Can you work these out from the model? Positions are in its coordinate system, mm. A direction names the side the tool comes from. Coordinates: 2 decimals unless noted, no trailing zeros. Write each loop counter-clockwise with the first axis right and the second up, starting at its lowest first coordinate (ties: lowest second). Pieces come first, ordered by that corner, then holes. Notation, with made-up numbers: (21.5, 69) - (27.5, 69) arc R16 cw to (27.5, 87) - close; hole circle Ø9 at (33, -13). An arc over 180 degrees is marked (long way). One line per question, with ' | ' between items. Start each with the question number.
from build123d import *

# Parameters (mm, degrees)
CUT_EXTRUDE_1_DEPTH = 4
SKETCH_3_R          = 15
SKETCH_3_R_2        = 14.3
CUT_EXTRUDE_3_DEPTH = 1.3


with BuildPart() as part:
    # 草图1 → 旋转1 (revolve)
    with BuildSketch(Plane.XY):
        Polygon((0, 0), (0, 17.5), (50, 17.5), (50, 20), (85, 20), (85, 60), (935, 60), (935, 20), (970, 20), (970, 17.5), (1111.3, 17.5), (1111.3, 15), (1154.3, 15), (1154.3, 0), align=None)
    revolve(axis=Axis((1154.3, 0, 0), (-1, 0, 0)))

    # 草图2 → 切除-拉伸1 (cut)
    with BuildSketch(Plane(origin=(0, 15, 0), x_dir=(1, 0, 0), z_dir=(0, 1, 0))):
        with BuildLine():
            Line((1121.3, 4), (1164.3, 4))
            Line((1164.3, 4), (1164.3, -4))
            Line((1164.3, -4), (1121.3, -4))
            ThreePointArc((1121.3, -4), (1117.3, 0), (1121.3, 4))
        make_face()
    extrude(amount=-CUT_EXTRUDE_1_DEPTH, mode=Mode.SUBTRACT)

    # 草图3 → 切除-拉伸3 (cut)
    with BuildSketch(Plane(origin=(1144.5, 0, 0), x_dir=(0, 0, -1), z_dir=(1, 0, 0))):
        with Locations(Location((0, 0, 0), (0, 0, 90))):
            Circle(SKETCH_3_R)
        Circle(SKETCH_3_R_2, mode=Mode.SUBTRACT)
    extrude(amount=-CUT_EXTRUDE_3_DEPTH, mode=Mode.SUBTRACT)


solid = part.part
(1) If we mould it in two halves opening along X, with no side actions, what happens to faces 4 (the face through (1144.5, -13.4, 5.6)), 5 (the face through (935, 26, -1)), 6 (the face through (1041.639, -13.887, 10.648))? For each: +X half, -X half, draft (parallel to the pull), parting line (faces both ways), or undercut.
(2) If we section it at B-B on x = 760.5: List the corners of the cut face in (y, z) for me, plus the area to 3 significant figures.
(3) If we section it at D-D on y = 49.5: List the corners of the cut face in (x, z) for me.
(4) Which directions (+Z, -Z, +X, -X, +Y, -Y) give clear straight access to the entire face, cutting with the end or side of a thin tool? Please do faces 1 (the face through (1143.2, -13.4, 5.6)), 2 (the face through (1127.473, -14.985, -0.66)), 3 (the face through (67.745, -4.336, 19.524)).
(5) If we section it at C-C on z = -42.5: List the corners of the cut face in (x, y) for me, plus the area to 3 significant figures.
(6) If I drill on probe 1 along X at (y, z) = (43.5, 13); probe 2 along Z at (x, y) = (619, -0.5); probe 3 along Y at (x, z) = (177.5, -4), over which ranges is the centre line in solid material (lowest first)?
(7) I'm going to push flat-ended pins straight in: pin 1 (3 mm diameter, centred on x = 1144, y = 12.5, fed in from +Z); pin 2 (1.5 mm diameter, centred on x = 171, y = -32.5, fed in from -Z); pin 3 (12 mm diameter, centred on x = 257, z = -16.5, fed in from +Y). Where does each tip first touch, or does it pass through?
Values:
1) face 4: undercut | face 5: +X half | face 6: draft
2) outline: circle Ø120 at (0, 0) | area: 11,300 mm2
3) outline: (85, -33.91) - (935, -33.91) - (935, 33.91) - (85, 33.91) - close
4) face 1: none | face 2: +X | face 3: -X
5) outline: (85, -42.35) - (935, -42.35) - (935, 42.35) - (85, 42.35) - close | area: 72,000 mm2
6) probe 1: 85 to 935 | probe 2: -60 to 60 | probe 3: -59.87 to 59.87
7) pin 1: z = 10.1 | pin 2: z = -50.91 | pin 3: y = 59.07
